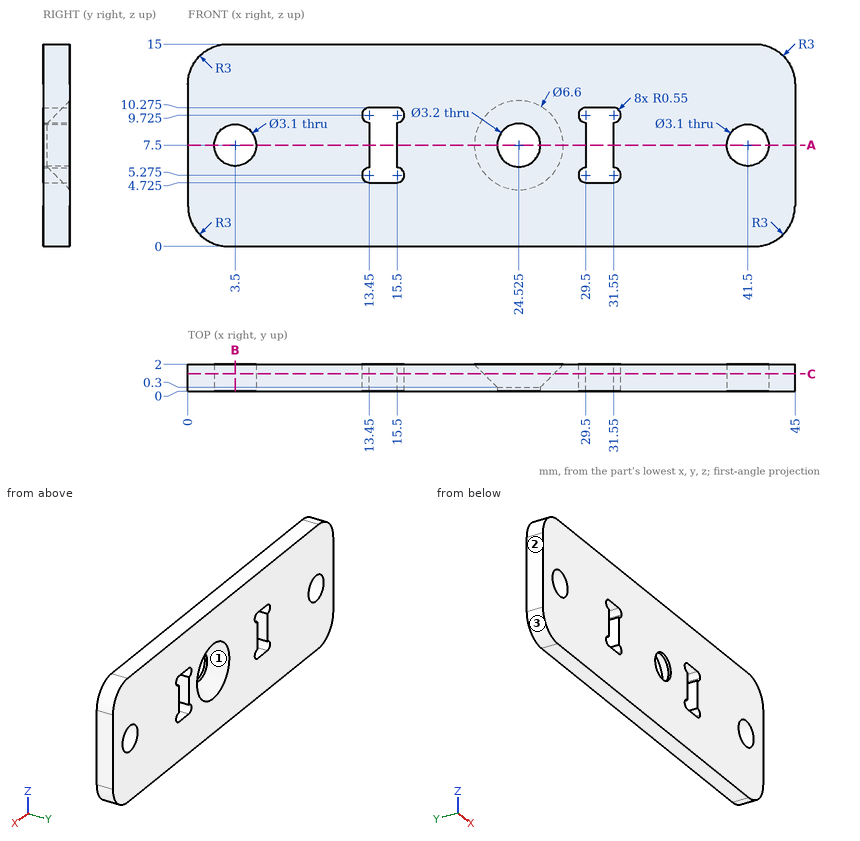
The figure shows three views and two pictorial views of one solid part (mm, origin at its lowest corner). Answer the questions. Round coordinates to 2 decimals unless told otherwise and drop trailing zeros. Write each loop counter-clockwise with the first axis right and the second up, starting at its lowest first coordinate (ties: lowest second). Pieces come first, ordered by that corner, then holes. Notation, with made-up numbers: (56, 73) -> (80, 73) arc R12 ccw to (80, 78) -> close; hole circle Ø4 at (-29, 6.25). An arc over 180 degrees is marked (long way). Answer as a JSON object with one key per item and string values. Group by question number.
Q1. Determine the mould class of the marked faces 1, 2 and 3 for opening direction Z: pulls with the +Z half, pulls with the -Z half, needs draft (parallel to the pull), parting line crosses it, or undercut.
Q2. Section C-C (y = 1.3) is taken. Write down the section's boundary in (x, z) (3 decimals), plus the area to 3 significant figures.
Q3. This flat-tipped pin is pushed along its axis until it touches: pin 1 Ø4 at (x, z) = (3.5, 7.5) entering from -Y. Where does it stop, or does it pass through?
Q4. Section B-B (x = 3.5) is taken. Write down the section's boundary in (y, z), plus the area to 3 significant figures.
Q5. Straight lines are drawn through the part: line 1 along X through (y, z) = (0.2, 7.5) (3 decimals); line 2 along Z through (x, y) = (32, 1.75); line 3 along X through (y, z) = (0.55, 7.5) (3 decimals). For each, find the intervals that lie inside material, in ascending order.
Q6. Section A-A (z = 7.5) is taken. Write down the section's boundary in (x, y) (3 decimals).
Check values:
{
 "1": {"face 1": "undercut", "face 2": "needs draft", "face 3": "pulls with the -Z half"},
 "2": {"outline": "(0, 3) arc R3 ccw to (3, 0) -> (42, 0) arc R3 ccw to (45, 3) -> (45, 12) arc R3 ccw to (42, 15) -> (3, 15) arc R3 ccw to (0, 12) -> close; hole circle Ø3.1 at (3.5, 7.5); hole (13.45, 4.725) -> (15.5, 4.725) arc R0.55 ccw to (15.5, 5.825) -> (15.5, 9.175) arc R0.55 ccw to (15.5, 10.275) -> (13.45, 10.275) arc R0.55 ccw to (13.45, 9.175) -> (13.45, 5.825) arc R0.55 ccw to start; hole circle Ø5.2 at (24.525, 7.5); hole (29.5, 4.725) -> (31.55, 4.725) arc R0.55 ccw to (31.55, 5.825) -> (31.55, 9.175) arc R0.55 ccw to (31.55, 10.275) -> (29.5, 10.275) arc R0.55 ccw to (29.5, 9.175) -> (29.5, 5.825) arc R0.55 ccw to start; hole circle Ø3.1 at (41.5, 7.5)", "area": "604 mm^2"},
 "3": {"pin 1": "y = 0"},
 "4": {"outline": "(0, 0) -> (2, 0) -> (2, 5.95) -> (0, 5.95) -> close; (0, 9.05) -> (2, 9.05) -> (2, 15) -> (0, 15) -> close", "area": "23.8 mm^2"},
 "5": {"line 1": "0 to 1.95, 5.05 to 13.45, 15.5 to 22.925, 26.125 to 29.5, 31.55 to 39.95, 43.05 to 45", "line 2": "0 to 4.96, 5.59 to 9.41, 10.04 to 15", "line 3": "0 to 1.95, 5.05 to 13.45, 15.5 to 22.675, 26.375 to 29.5, 31.55 to 39.95, 43.05 to 45"},
 "6": {"outline": "(0, 0) -> (1.95, 0) -> (1.95, 2) -> (0, 2) -> close; (5.05, 0) -> (13.45, 0) -> (13.45, 2) -> (5.05, 2) -> close; (15.5, 0) -> (22.925, 0) -> (22.925, 0.3) -> (21.225, 2) -> (15.5, 2) -> close; (26.125, 0) -> (29.5, 0) -> (29.5, 2) -> (27.825, 2) -> (26.125, 0.3) -> close; (31.55, 0) -> (39.95, 0) -> (39.95, 2) -> (31.55, 2) -> close; (43.05, 0) -> (45, 0) -> (45, 2) -> (43.05, 2) -> close"}
}
